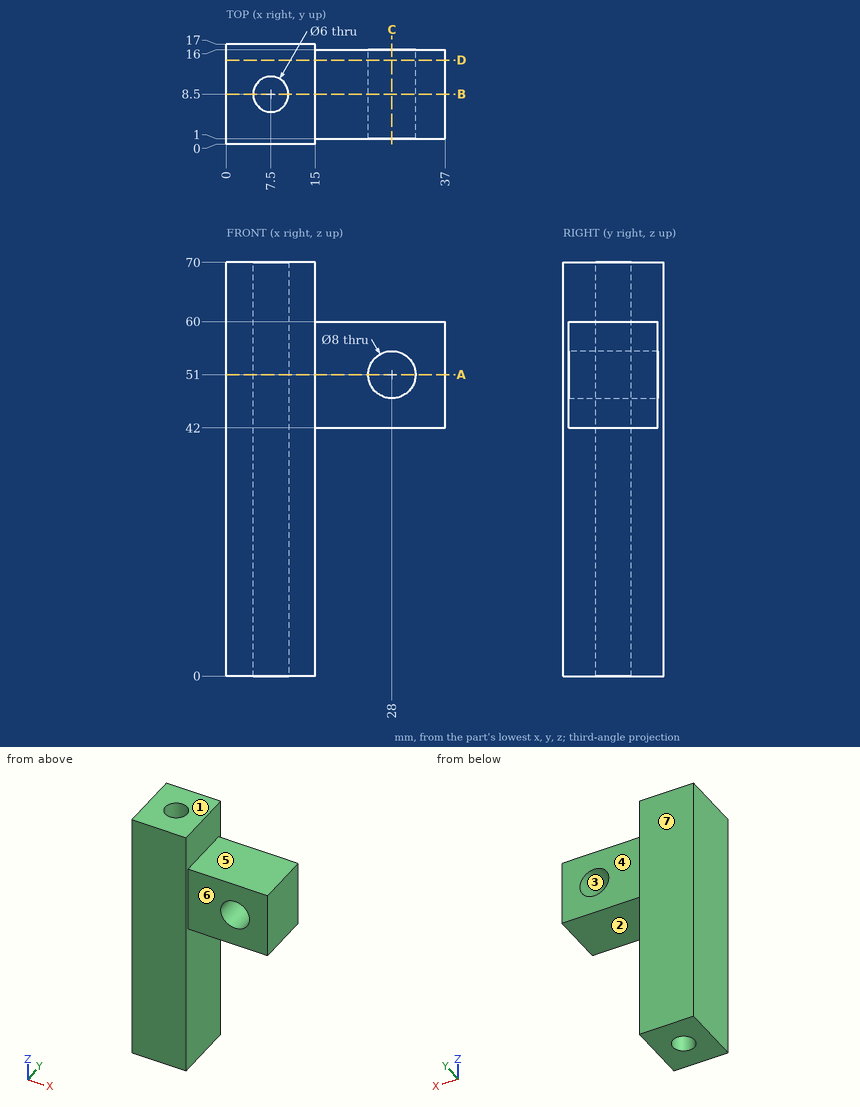
Could you check a few things on this drawing? It's one solid part, dimensions in mm from its lowest x, y, z. A direction names the side the tool comes from. Coordinates: 2 decimals unless noted, no trailing zeros. Loops run counter-clockwise (first coordinate to the right, second up) from the corner with the lowest first, then second, coordinate; pieces in that order, holes last. Notation, with made-up numbers: (-16, -39) - (21, -39) arc R33 cw to (21, -1) - close; hole circle Ø2 at (-16, 81). An arc over 180 degrees is marked (long way). Answer as a JSON object with one key per item and string values. Group by question number.
Item 1: If we section it at C-C (x = 28): List the corners of the cut face in (y, z) for me, plus the area to 3 significant figures.
Item 2: If we mould it in two halves opening along Z, with no side actions, what happens to the marked faces 1, 2 and 3? For each: released by +Z, released by -Z, zero draft, split by the parting line, or undercut.
Item 3: On a 3-axis mill with a long thin cutter (end or side, diameter ignored), from which of +Z, -Z, +X, -X, +Y, -Y can I reach the whole of each face in a straight line? I mean the marked faces 4, 5, 6 and 7. Say none if no direction works.
Item 4: For pin 1 (2 mm diameter, centred on x = 30, y = 13.5, fed in from +Z); pin 2 (5 mm diameter, centred on x = 21.5, z = 41, fed in from +Y); pin 3 (10 mm diameter, centred on x = 24, z = 52, fed in from -Y), each with a flat end and sliding along its axis, tell me the tip position at first contact or that it passes through.
Item 5: If we section it at B-B (y = 8.5): List the corners of the cut face in (x, z) for me, plus the area to 3 significant figures.
Item 6: If we section it at D-D (y = 14.25): List the corners of the cut face in (x, z) for me, plus the area to 3 significant figures.
Item 7: If I drill on L1, parallel to Y at x = 7.5, z = 31; L2, parallel to Z at x = 31, y = 12.25; L3, parallel to X at y = 10.5, z = 29, over which ranges is the centre line in solid material (lowest first)? Write a range as from..to.
Item 8: If we section it at A-A (z = 51): List the corners of the cut face in (x, y) for me, plus the area to 3 significant figures.
Returned:
{
 "1": {"outline": "(1, 42) - (16, 42) - (16, 47) - (1, 47) - close; (1, 55) - (16, 55) - (16, 60) - (1, 60) - close", "area": "150 mm²"},
 "2": {"face 1": "released by +Z", "face 2": "released by -Z", "face 3": "undercut"},
 "3": {"face 4": "+Z, -Z, +X, +Y", "face 5": "+Z, +X, +Y, -Y", "face 6": "+Z, -Z, +X, -Y", "face 7": "+Z, -Z, +X, -X, +Y"},
 "4": {"pin 1": "stops at z = 60", "pin 2": "stops at y = 16", "pin 3": "stops at y = 1"},
 "5": {"outline": "(0, 0) - (4.5, 0) - (4.5, 70) - (0, 70) - close; (10.5, 0) - (15, 0) - (15, 42) - (37, 42) - (37, 60) - (15, 60) - (15, 70) - (10.5, 70) - close; hole circle Ø8 at (28, 51)", "area": "976 mm²"},
 "6": {"outline": "(0, 0) - (15, 0) - (15, 42) - (37, 42) - (37, 60) - (15, 60) - (15, 70) - (0, 70) - close; hole circle Ø8 at (28, 51)", "area": "1,400 mm²"},
 "7": {"L1": "y = 0..5.5, 11.5..17", "L2": "z = 42..48.35, 53.65..60", "L3": "x = 0..5.26, 9.74..15"},
 "8": {"outline": "(0, 0) - (15, 0) - (15, 1) - (24, 1) - (24, 16) - (15, 16) - (15, 17) - (0, 17) - close; (32, 1) - (37, 1) - (37, 16) - (32, 16) - close; hole circle Ø6 at (7.5, 8.5)", "area": "437 mm²"}
}
